from build123d import *

# Parameters (mm, degrees)
EXTRUDE_1_DEPTH     = 20
FILLET_1_R          = 1
SKETCH_2_R          = 3
CUT_EXTRUDE_1_DEPTH = 50.889878733


with BuildPart() as part:
    # 草图1 → 凸台-拉伸1 (new body)
    with BuildSketch(Plane.XY):
        with BuildLine():
            Line((0, 0), (12, 0))
            Line((12, 0), (12, 8))
            Line((12, 8), (33, 8))
            Line((33, 8), (33, 0))
            Line((33, 0), (45, 0))
            Line((45, 0), (45, -5))
            Line((45, -5), (30, -5))
            Line((30, -5), (30, -2))
            ThreePointArc((30, -2), (22.5, 5.5), (15, -2))
            Line((15, -2), (15, -5))
            Line((15, -5), (0, -5))
            Line((0, -5), (0, 0))
        make_face()
    extrude(amount=EXTRUDE_1_DEPTH)

    # 圆角1
    fillet_1_edges = [part.edges().sort_by_distance(p)[0] for p in [
        (12, 8, 10),
        (33, 8, 10),
    ]]
    fillet(fillet_1_edges, radius=FILLET_1_R)

    # 草图2 → 切除-拉伸1 (cut, through all)
    with BuildSketch(Plane(origin=(0, 0, 0), x_dir=(1, 0, 0), z_dir=(0, 1, 0))):
        with Locations(Location((5.5, -10, 0), (0, 0, 270))):
            Circle(SKETCH_2_R)
        with Locations(Location((39.5, -10, 0), (0, 0, 270))):
            Circle(SKETCH_2_R)
    extrude(amount=-CUT_EXTRUDE_1_DEPTH, mode=Mode.SUBTRACT)


solid = part.part
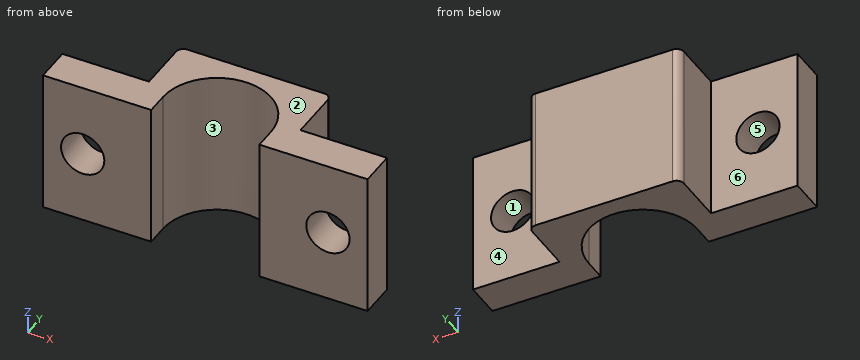
Model file for the job. Use its own axes, mm. Face numbers are marked on the shaded views. A direction names the side the tool comes from. Round coordinates to 2 decimals unless told otherwise and drop trailing zeros. Order: outer loops, then holes, each group sorted by start corner. A loop starts at its lowest first (then second) coordinate and runs counter-clockwise, first axis right, second up.
(1) Drill centre lines: line 1 (X direction, y = -2.6, z = 10); line 2 (X direction, y = -1.1, z = 10); line 3 (X direction, y = -3.5, z = 13.25). Where is each one in solid material? Low to high.
(2) Band-saw the part on B-B (x = 5.5). List the corners of the cut face in (y, z).
(3) Pin check, flat tips, straight feed: pin 1 (5.5 mm diameter, centred on x = 39.5, z = 10, fed in from +Y); pin 2 (2 mm diameter, centred on y = -3, z = 4, fed in from -X); pin 3 (1 mm diameter, centred on y = 2.5, z = 17.5, fed in from +X); pin 4 (9.5 mm diameter, centred on x = 41.5, z = 12, fed in from +Y). Stop position of each tip, or through.
(4) 3-axis set-ups, long thin cutter, end or side, ignore diameter. For the marked faces 4, 5 and 6: which of +Z, -Z, +X, -X, +Y, -Y reach the whole face in a straight line?
(5) Band-saw the part on D-D (y = 1.25). List the corners of the cut face in (x, z), then the cut area to 3 significant figures.
(6) Band-saw the part on C-C (z = 10). List the corners of the cut face in (x, y).
(7) Band-saw the part on A-A (y = -4). List the corners of the cut face in (x, z), then the cut area to 3 significant figures.
(8) Pull direction Z, two halves, no side cores. Call the marked faces 1, 2 and 3: released by +Z, released by -Z, zero draft, split by the parting line, or undercut.
Verdict:
1. line 1: x = 0 to 2.5, 8.5 to 15, 30 to 36.5, 42.5 to 45
1. line 2: x = 0 to 2.5, 8.5 to 15.05, 29.95 to 36.5, 42.5 to 45
1. line 3: x = 0 to 15, 30 to 45
2. outline: (-5, 0) - (0, 0) - (0, 7) - (-5, 7) - close; (-5, 13) - (0, 13) - (0, 20) - (-5, 20) - close
3. pin 1: passes through
3. pin 2: stops at x = 0
3. pin 3: stops at x = 33
3. pin 4: stops at y = 0
4. face 4: +Z, -Z, +X, +Y
4. face 5: +Y, -Y
4. face 6: +Z, -Z, -X, +Y
5. outline: (12, 0) - (15.74, 0) - (15.74, 20) - (12, 20) - close; (29.26, 0) - (33, 0) - (33, 20) - (29.26, 20) - close
5. area: 150 mm2
6. outline: (0, -5) - (2.5, -5) - (2.5, 0) - (0, 0) - close; (8.5, -5) - (15, -5) - (15, -2) arc R7.5 cw to (30, -2) - (30, -5) - (36.5, -5) - (36.5, 0) - (33, 0) - (33, 7) arc R1 ccw to (32, 8) - (13, 8) arc R1 ccw to (12, 7) - (12, 0) - (8.5, 0) - close; (42.5, -5) - (45, -5) - (45, 0) - (42.5, 0) - close
7. outline: (0, 0) - (15, 0) - (15, 20) - (0, 20) - close; (30, 0) - (45, 0) - (45, 20) - (30, 20) - close; hole circle Ø6 at (5.5, 10); hole circle Ø6 at (39.5, 10)
7. area: 543 mm2
8. face 1: undercut
8. face 2: released by +Z
8. face 3: zero draft
